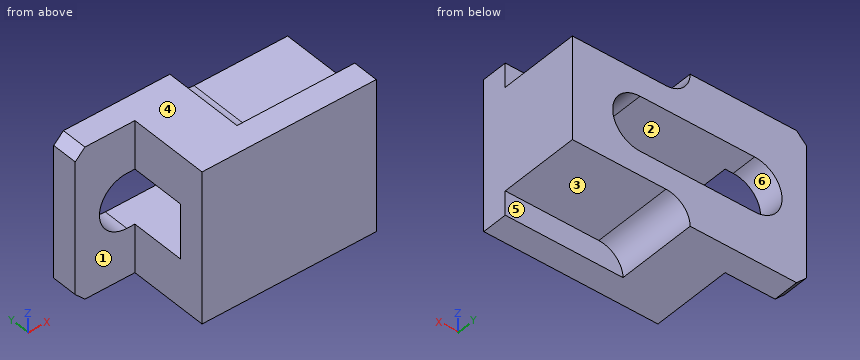
```python
from build123d import *

# Parameters (mm, degrees)
BASE_BLOCK_DEPTH       = 47
SIDE_NOTCH_A_DEPTH     = 25
SIDE_NOTCH_B_DEPTH     = 25
GUIDE_SLOT_DEPTH       = 25
EDGE_CHAMFER_3X45_SIZE = 3


with BuildPart() as part:
    # Base Profile Sketch → Base Block (new body)
    with BuildSketch(Plane.XY):
        Polygon((0, 0), (54, 0), (54, 8), (54, 33), (-18.5, 33), (-18.5, 25), (0, 25), align=None)
    extrude(amount=-BASE_BLOCK_DEPTH)

    # Side Notch A Sketch → Side Notch A (cut)
    with BuildSketch(Plane(origin=(0, 33, 0), x_dir=(1, 0, 0), z_dir=(0, 1, 0))):
        with BuildLine():
            Line((54, 0), (54, 7.5))
            Line((54, 7.5), (25, 7.5))
            ThreePointArc((25, 7.5), (19.696699141, 5.303300859), (17.5, 0))
            Line((17.5, 0), (25, 0))
            Line((25, 0), (54, 0))
        make_face()
    extrude(amount=-SIDE_NOTCH_A_DEPTH, mode=Mode.SUBTRACT)

    # Side Notch B Sketch → Side Notch B (cut)
    with BuildSketch(Plane(origin=(0, 33, 0), x_dir=(1, 0, 0), z_dir=(0, 1, 0))):
        with BuildLine():
            Line((54, 47), (54, 39.5))
            Line((54, 39.5), (25, 39.5))
            ThreePointArc((25, 39.5), (19.696699141, 41.696699141), (17.5, 47))
            Line((17.5, 47), (25, 47))
            Line((25, 47), (54, 47))
        make_face()
    extrude(amount=-SIDE_NOTCH_B_DEPTH, mode=Mode.SUBTRACT)

    # Guide Slot Sketch → Guide Slot (cut)
    with BuildSketch(Plane(origin=(0, 33, 0), x_dir=(1, 0, 0), z_dir=(0, 1, 0))):
        with BuildLine():
            Line((-2.5, 32), (33, 32))
            ThreePointArc((33, 32), (41.5, 23.5), (33, 15))
            Line((33, 15), (-2.5, 15))
            ThreePointArc((-2.5, 15), (-11, 23.5), (-2.5, 32))
        make_face()
    extrude(amount=-GUIDE_SLOT_DEPTH, mode=Mode.SUBTRACT)

    # Edge Chamfer 3x45
    edge_chamfer_3x45_edges = [part.edges().sort_by_distance(p)[0] for p in [
        (-18.5, 29, -47),
        (-18.5, 29, 0),
    ]]
    chamfer(edge_chamfer_3x45_edges, length=EDGE_CHAMFER_3X45_SIZE)


solid = part.part
```
Work out the finished part from the listing and answer in its coordinate system (mm). Face numbers are marked on the shaded views. A direction names the side the tool comes from. Round coordinates to 2 decimals unless told otherwise and drop trailing zeros. Order: outer loops, then holes, each group sorted by start corner. A loop starts at its lowest first (then second) coordinate and runs counter-clockwise, first axis right, second up.
Q1. The mould has two halves that part along Z. Classify the marked faces 4, 5 and 6: pulls with the +Z half, pulls with the -Z half, needs draft (parallel to the pull), parting line crosses it, or undercut.
Solution:
face 4: pulls with the +Z half
face 5: needs draft
face 6: undercut
Q2. A cutting plane is placed at B-B, the plane y = 21. Determine the outline of the cut face in (x, z).
Solution:
outline: (0, -47) - (17.5, -47) arc R7.5 cw to (25, -39.5) - (54, -39.5) - (54, -7.5) - (25, -7.5) arc R7.5 cw to (17.5, 0) - (0, 0) - (0, -15) - (33, -15) arc R8.5 cw to (33, -32) - (0, -32) - close
Q3. Given pin 1 Ø12.5 at (x, y) = (38.5, 19.5) entering from +Z; pin 2 Ø4 at (x, y) = (40.5, 13.5) entering from -Z; pin 3 Ø2 at (y, z) = (18, -20.5) entering from -X; pin 4 Ø6 at (x, z) = (33.5, -41.5) entering from +Y, each flat-ended and moving along its own axis, determine where each tip first touches the part or whether it passes through.
Solution:
pin 1: stops at z = -7.5
pin 2: stops at z = -39.5
pin 3: stops at x = 40.5
pin 4: stops at y = 33
Q4. A cutting plane is placed at A-A, the plane z = -23.5. Determine the outline of the cut face in (x, y), then the cut area to 4 significant figures.
Solution:
outline: (-18.5, 25) - (-11, 25) - (-11, 33) - (-18.5, 33) - close; (0, 0) - (54, 0) - (54, 33) - (41.5, 33) - (41.5, 8) - (0, 8) - close
area: 804.5 mm2
Q5. A tool of negligible diameter and unlimited length cuts with its end or side. For the marked faces 1, 2 and 3, from which of +Z, -Z, +X, -X, +Y, -Y can it reach the whole face along a straight path? Write none if from no direction.
Solution:
face 1: +Z, -Z, -X, -Y
face 2: +Y
face 3: -Z, +X, +Y
Q6. A cutting plane is placed at C-C, the plane z = -6. Determine the outline of the cut face in (x, y).
Solution:
outline: (-18.5, 25) - (0, 25) - (0, 0) - (54, 0) - (54, 8) - (20.5, 8) - (20.5, 33) - (-18.5, 33) - close
Q7. A cutting plane is placed at D-D, the plane x = 21. Determine the outline of the cut face in (y, z), then the cut area to 3 significant figures.
Solution:
outline: (0, -47) - (8, -47) - (8, -40.66) - (33, -40.66) - (33, -32) - (8, -32) - (8, -15) - (33, -15) - (33, -6.34) - (8, -6.34) - (8, 0) - (0, 0) - close
area: 809 mm2
Q8. Find the intervals of material crossed by line 1 along Z through (x, y) = (5, 11.5); line 2 along Z through (x, y) = (26, 10.5); line 3 along Z through (x, y) = (42.5, 27), in increasing order.
Solution:
line 1: z = -47 to -32, -15 to 0
line 2: z = -39.5 to -32, -15 to -7.5
line 3: z = -39.5 to -7.5
